For this review, take the finished solid that the model builds, in its own axes (mm). A direction names the side the tool comes from. Coordinates: 2 decimals unless noted, no trailing zeros. Order: outer loops, then holes, each group sorted by start corner. A loop starts at its lowest first (then second) coordinate and runs counter-clockwise, first axis right, second up. Notation, with made-up numbers: (89, 41.25) -> (108, 41.25) arc R7 cw to (108, 49.25) -> close; hole circle Ø4 at (88, -37.5). An arc over 180 degrees is marked (long way). Write item = value, one per line. Start each with the question number.
1) Consider section D-D on y = 4.75. Give the boundary of the cut face in (x, z).
2) Consider section A-A on x = -3. Give the boundary of the cut face in (y, z).
3) Insertion check: pin 1 Ø5 at (x, z) = (14, -3.5) entering from -Y; pin 2 Ø4 at (x, y) = (-6, 4.5) entering from +Z; pin 3 Ø2 at (x, z) = (-6, 5.5) entering from +Y. Each pin has a flat end and moves straight along its axis. Give the tip position at first contact, or say it passes through.
4) Draft analysis for pull direction Z (two halves, no side actions). For faces 6 (the face through (-12.43, 2.59, -2.85)), 7 (the face through (0, -4, 3)), 8 (the face through (16, -7, 6)), state which applies: +Z half, -Z half, draft (parallel to the pull), parting line (faces both ways), or undercut.
5) Wall thickness on probe 1 along X at (y, z) = (-5.55, 4.6); probe 2 along Z at (x, y) = (-14, -5.75); probe 3 along X at (y, z) = (-6.5, -6): over which ranges is each line inside the solid? List them lowest first. Write a range as [from, to].
6) Consider section B-B on y = 1. Give the boundary of the cut face in (x, z).
7) Machinability: for faces 1 (the face through (-16, -7, 6)), 2 (the face through (-17.5, 0, -3)), 3 (the face through (12, -4, -4)), 4 (the face through (-10.89, -5.52, 5.93)), 5 (the face through (0, 2, 0.5)), which of the approach directions +Z, -Z, +X, -X, +Y, -Y give a long, thin tool a straight path to every point of the face, cutting with its end or side? Answer none if there is none.
8) Consider section C-C on z = -3. Give the boundary of the cut face in (x, y), and give its area (3 significant figures).
from build123d import *

# Parameters (mm, degrees)
SKETCH1_W                                            = 35
SKETCH1_H                                            = 18
BOSS_EXTRUDE1_DEPTH                                  = 7.5
SKETCH2_W                                            = 7
SKETCH2_H                                            = 13
CUT_EXTRUDE1_DEPTH                                   = 37.908671068
F_5_0_5_DIAMETER_HOLE1_D                             = 5
F_3_0_3_DIAMETER_HOLE2_D                             = 3
F_3_0_3_DIAMETER_HOLE2_DEPTH                         = 3
F_3_0_3_DIAMETER_HOLE2_TIP                           = 0.901290929
M3_TAPPED_HOLE1_D                                    = 2.5
HOLE_SIZE_PER_SOCKET_HEAD_CAP_SCREW_TYPE_D           = 3.4
HOLE_SIZE_PER_SOCKET_HEAD_CAP_SCREW_TYPE_CBORE_D     = 6
HOLE_SIZE_PER_SOCKET_HEAD_CAP_SCREW_TYPE_CBORE_DEPTH = 5
CHAMFER1_SIZE                                        = 3


with BuildPart() as part:
    # Sketch1 → Boss-Extrude1 (new, symmetric)
    with BuildSketch(Plane.XY):
        Rectangle(SKETCH1_W, SKETCH1_H)
    extrude(amount=BOSS_EXTRUDE1_DEPTH, both=True)

    # Sketch2 → Cut-Extrude1 (cut, through all)
    with BuildSketch(Plane(origin=(17.5, 0, 0), x_dir=(0, 0, -1), z_dir=(1, 0, 0))):
        with Locations((-4, 2.5)):
            Rectangle(SKETCH2_W, SKETCH2_H)
    extrude(amount=-CUT_EXTRUDE1_DEPTH, mode=Mode.SUBTRACT)

    # Ø5.0 (5) Diameter Hole1 (through all)
    with Locations(Plane.XY.offset(0.5)):
        with Locations((-5, 1), (5, 1)):
            Hole(F_5_0_5_DIAMETER_HOLE1_D / 2)

    # Ø3.0 (3) Diameter Hole2
    with Locations(Plane(origin=(0, -4, 0), x_dir=(1, 0, 0), z_dir=(0, 1, 0))):
        with Locations((10.2, -4.6), (-10.2, -4.6)):
            Hole(F_3_0_3_DIAMETER_HOLE2_D / 2, depth=F_3_0_3_DIAMETER_HOLE2_DEPTH)
            with Locations((0, 0, -(F_3_0_3_DIAMETER_HOLE2_DEPTH + F_3_0_3_DIAMETER_HOLE2_TIP / 2))):  # 118° drill point
                Cone(0, F_3_0_3_DIAMETER_HOLE2_D / 2, F_3_0_3_DIAMETER_HOLE2_TIP, mode=Mode.SUBTRACT)

    # M3 Tapped Hole1 (through all)
    with Locations(Plane(origin=(0, -9, 0), x_dir=(-1, 0, 0), z_dir=(0, -1, 0))):
        with Locations((0, -4.6)):
            Hole(M3_TAPPED_HOLE1_D / 2)

    # Hole size per socket head cap screw type1 (through all)
    with Locations(Plane(origin=(0, -9, 0), x_dir=(-1, 0, 0), z_dir=(0, -1, 0))):
        with Locations((14, 3.5), (-14, 3.5)):
            CounterBoreHole(HOLE_SIZE_PER_SOCKET_HEAD_CAP_SCREW_TYPE_D / 2, HOLE_SIZE_PER_SOCKET_HEAD_CAP_SCREW_TYPE_CBORE_D / 2, HOLE_SIZE_PER_SOCKET_HEAD_CAP_SCREW_TYPE_CBORE_DEPTH)

    # Chamfer1
    chamfer1_edges = [part.edges().sort_by_distance(p)[0] for p in [
        (-17.5, -6.5, 7.5),
        (17.5, -6.5, 7.5),
    ]]
    chamfer(chamfer1_edges, length=CHAMFER1_SIZE)


solid = part.part
Answer sheet:
q1.outline = (-17.5, -7.5) -> (17.5, -7.5) -> (17.5, 0.5) -> (-17.5, 0.5) -> close; hole circle Ø3.4 at (-14, -3.5); hole circle Ø3.4 at (14, -3.5)
q2.outline = (-9, -7.5) -> (-0.5, -7.5) -> (-0.5, 0.5) -> (-4, 0.5) -> (-4, 7.5) -> (-9, 7.5) -> close; (2.5, -7.5) -> (9, -7.5) -> (9, 0.5) -> (2.5, 0.5) -> close
q3.pin_1 = -4
q3.pin_2 = 0.5
q3.pin_3 = -4
q4.face_6 = undercut
q4.face_7 = draft
q4.face_8 = +Z half
q5.probe_1 = [-17.4, -11.7], [-8.7, -1.25], [1.25, 8.7], [11.7, 17.4]
q5.probe_2 = [-7.5, -6.5], [-0.5, 7.5]
q5.probe_3 = [-17.5, -15.66], [-12.34, 12.34], [15.66, 17.5]
q6.outline = (-17.5, -7.5) -> (-7.5, -7.5) -> (-7.5, 0.5) -> (-17.5, 0.5) -> close; (-2.5, -7.5) -> (2.5, -7.5) -> (2.5, 0.5) -> (-2.5, 0.5) -> close; (7.5, -7.5) -> (17.5, -7.5) -> (17.5, 0.5) -> (7.5, 0.5) -> close; hole circle Ø3.4 at (-14, -3.5); hole circle Ø3.4 at (14, -3.5)
q7.face_1 = +Z, -X, +Y, -Y
q7.face_2 = +Z, -Z, -X, +Y, -Y
q7.face_3 = -Y
q7.face_4 = +Y
q7.face_5 = +Z, +X, -X, +Y
q8.outline = (-17.5, -9) -> (-16.96, -9) -> (-16.96, -4) -> (-15.62, -4) -> (-15.62, 9) -> (-17.5, 9) -> close; (-12.38, -4) -> (-11.04, -4) -> (-11.04, -9) -> (11.04, -9) -> (11.04, -4) -> (12.38, -4) -> (12.38, 9) -> (-12.38, 9) -> close; (15.62, -4) -> (16.96, -4) -> (16.96, -9) -> (17.5, -9) -> (17.5, 9) -> (15.62, 9) -> close; hole circle Ø5 at (-5, 1); hole circle Ø5 at (5, 1)
q8.area = 447 mm2
